Here's how the part is built. I have some questions about the finished solid (model axes, mm). Face numbers are marked on the shaded views. A direction names the side the tool comes from. Round coordinates to 2 decimals unless told otherwise and drop trailing zeros. Order: outer loops, then holes, each group sorted by start corner. A loop starts at its lowest first (then second) coordinate and runs counter-clockwise, first axis right, second up. Notation, with made-up numbers: (-20, 38.25) -> (2, 38.25) arc R12 cw to (2, 47.25) -> close; hole circle Ø5 at (-23.5, -11). An arc over 180 degrees is marked (long way). Use a Markdown table: item, result. Add a question column.
(1) I want a section at A-A, the plane x = 14. Please give me the cut outline in (y, z), then the cut area to 3 significant figures.
(2) I want a section at B-B, the plane x = 6.75. Please give me the cut outline in (y, z).
(3) On a 3-axis mill with a long thin cutter (end or side, diameter ignored), from which of +Z, -Z, +X, -X, +Y, -Y can I reach the whole of each face in a straight line? I mean the marked faces 4 and 5. Say none if no direction works.
(4) I'm going to push flat-ended pins straight in: P1, Ø3, axis at y = -0.5, z = -1, coming from the -X side; P2, Ø2.5, axis at x = 14.5, z = 0, coming from the +Y side; P3, Ø2, axis at x = 10.5, z = -0.5, coming from the -Y side; P4, Ø2, axis at x = 8.5, y = -1, coming from the -Z side. Where does each tip first touch, or does it pass through?
(5) Thinking about a two-plate mould opening in Z: for the marked faces 1, 2 and 3, which applies, pulls with the +Z half, pulls with the -Z half, needs draft (parallel to the pull), parting line crosses it, or undercut?
(6) If I drill on probe 1 along X at (y, z) = (0.25, 0); probe 2 along Y at (x, z) = (7.5, 0); probe 3 along Z at (x, y) = (14.5, -0.6), over which ranges is the centre line in solid material (lowest first)?
from build123d import *

# Parameters (mm, degrees)
FILLET_1_R          = 0.5
CHAMFER_1_SIZE      = 0.866025404
CHAMFER_1_SIZE2     = 0.5
SKETCH_2_R          = 0.87
CUT_EXTRUDE_1_DEPTH = 500


with BuildPart() as part:
    # 草图1 → Revolve 700 (revolve)
    with BuildSketch(Plane.XY, mode=Mode.PRIVATE) as revolve_700_sk:
        with BuildLine():
            Line((0, 0), (17.5, 0))
            Line((17.5, 0), (17.5, 2))
            Line((17.5, 2), (1.5, 2))
            Line((1.5, 2), (1.5, 2.25))
            ThreePointArc((1.5, 2.25), (0.75, 3), (0, 2.25))
            Line((0, 2.25), (0, 0))
        make_face()
    revolve(revolve_700_sk.sketch.rotate(Axis((0, 0, 0), (1, 0, 0)), 90), axis=Axis((0, 0, 0), (1, 0, 0)))

    # 圆角1
    fillet_1_edges = [part.edges().sort_by_distance(p)[0] for p in [
        (1.5, 0, -2),
    ]]
    fillet(fillet_1_edges, radius=FILLET_1_R)

    # 倒角1
    chamfer_1_edges = [part.edges().sort_by_distance(p)[0] for p in [
        (17.5, 0, -2),
    ]]
    chamfer_1_side = [part.faces().sort_by_distance(p)[0] for p in [
        (9.737372436, 0, -2),
    ]]
    chamfer(chamfer_1_edges, length=CHAMFER_1_SIZE, length2=CHAMFER_1_SIZE2, reference=chamfer_1_side[0])

    # 草图2 → 切除-拉伸1 (cut, symmetric)
    with BuildSketch(Plane(origin=(0, 0, 0), x_dir=(1, 0, 0), z_dir=(0, 1, 0))):
        with Locations(Location((14.5, 0, 0), (0, 0, 270))):
            Circle(SKETCH_2_R)
    extrude(amount=CUT_EXTRUDE_1_DEPTH, both=True, mode=Mode.SUBTRACT)


solid = part.part
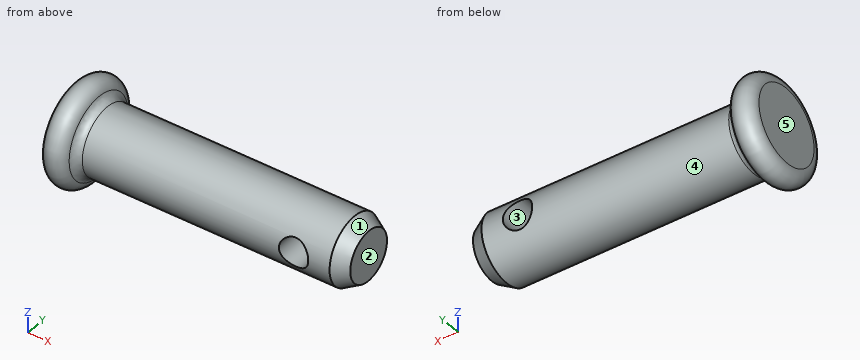
Taken from the geometry:
| question | item | result |
|---|---|---|
| 1 | outline | (-1.87, -0.71) arc R2 ccw to (1.87, -0.71) -> close; (-1.87, 0.71) -> (1.87, 0.71) arc R2 ccw to start |
| 1 | area | 6.99 mm2 |
| 2 | outline | circle Ø4 at (0, 0) |
| 3 | face 4 | +X |
| 3 | face 5 | +Z, -Z, -X, +Y, -Y |
| 4 | P1 | stops at x = 0 |
| 4 | P2 | stops at y = 2 |
| 4 | P3 | stops at y = -2 |
| 4 | P4 | stops at z = -2 |
| 5 | face 1 | parting line crosses it |
| 5 | face 2 | needs draft |
| 5 | face 3 | undercut |
| 6 | probe 1 | x = 0 to 13.63, 15.37 to 17.5 |
| 6 | probe 2 | y = -2 to 2 |
| 6 | probe 3 | z = -1.91 to -0.87, 0.87 to 1.91 |
